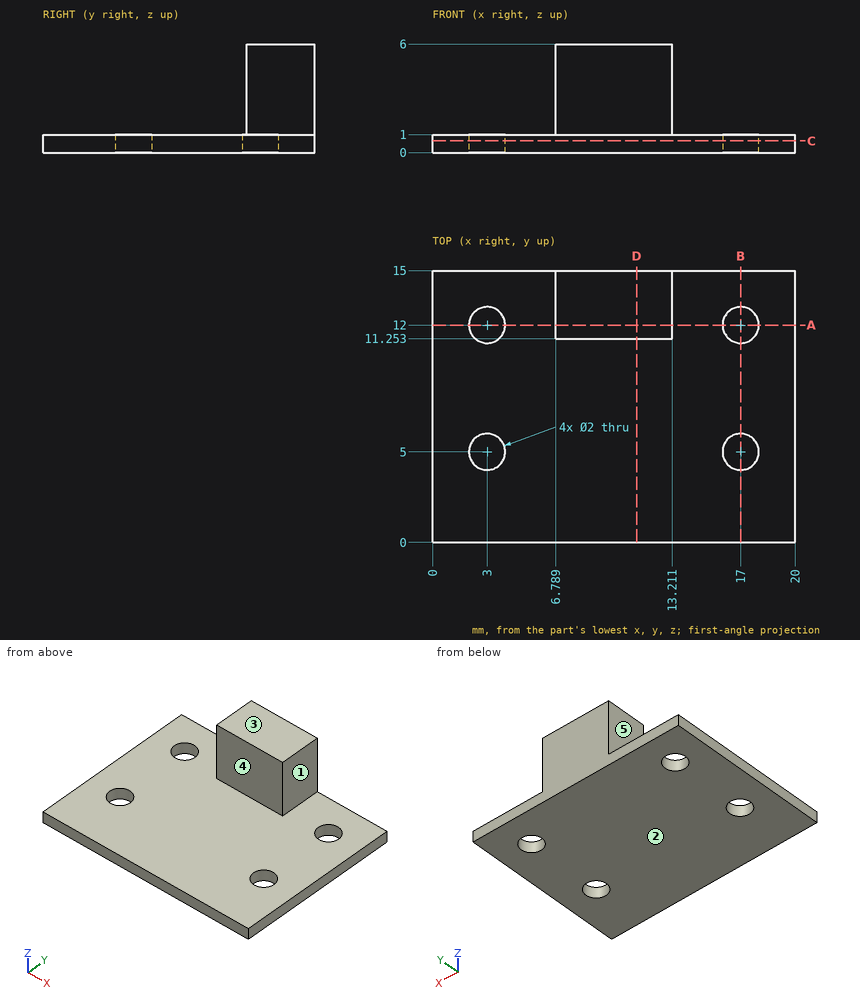
Input: dimensioned drawing with shaded views. Units: mm. Origin: part minimum x, y, z. A direction names the side the tool comes from. Round coordinates to 2 decimals unless told otherwise and drop trailing zeros. Order: outer loops, then holes, each group sorted by start corner. A loop starts at its lowest first (then second) coordinate and runs counter-clockwise, first axis right, second up. Notation, with made-up numbers: (48.5, -35.5) -> (53.5, -35.5) arc R8 cw to (53.5, -31.5) -> close; hole circle Ø7 at (55.5, 41). An arc over 180 degrees is marked (long way). Put each result on its own line as item: value. Start each with the question number.
Q1. First-contact query: pin 1 (1.5 mm diameter, centred on x = 11, z = 3, fed in from -Y); pin 2 (7.5 mm diameter, centred on x = 13, y = 5, fed in from +Z); pin 3 (1.1 mm diameter, centred on y = 13, z = 4, fed in from -X); pin 4 (1.2 mm diameter, centred on x = 17, y = 12, fed in from -Z) (3 decimals). Flat tips, straight axial feed; report the tip coordinate or a pass-through.
Q2. Section D-D on x = 11.25. Return the cut outline in (y, z).
Q3. Line query: probe 1 along Y at (x, z) = (17, 0.65); probe 2 along Z at (x, y) = (11.5, 5.25); probe 3 along Y at (x, z) = (11, 1.15). Output: solid intervals per line, ascending.
Q4. Reachability of the marked faces 1, 2, 3, 4 and 5 from +Z, -Z, +X, -X, +Y, -Y: full face, straight path, thin tool, end or side. Return the list, or none.
Q5. Section A-A on y = 12. Return the cut outline in (x, z).
Q6. Section B-B on x = 17. Return the cut outline in (y, z), and give its area (3 significant figures).
Q7. Section C-C on z = 0.65. Return the cut outline in (x, y).
Ans:
1. pin 1: stops at y = 11.25
1. pin 2: stops at z = 1
1. pin 3: stops at x = 6.79
1. pin 4: passes through
2. outline: (0, 0) -> (15, 0) -> (15, 6) -> (11.25, 6) -> (11.25, 1) -> (0, 1) -> close
3. probe 1: y = 0 to 4, 6 to 11, 13 to 15
3. probe 2: z = 0 to 1
3. probe 3: y = 11.25 to 15
4. face 1: +Z, +X, +Y, -Y
4. face 2: -Z, +X, -X, +Y, -Y
4. face 3: +Z, +X, -X, +Y, -Y
4. face 4: +Z, +X, -X, -Y
4. face 5: +Z, -X, +Y, -Y
5. outline: (0, 0) -> (2, 0) -> (2, 1) -> (0, 1) -> close; (4, 0) -> (16, 0) -> (16, 1) -> (13.21, 1) -> (13.21, 6) -> (6.79, 6) -> (6.79, 1) -> (4, 1) -> close; (18, 0) -> (20, 0) -> (20, 1) -> (18, 1) -> close
6. outline: (0, 0) -> (4, 0) -> (4, 1) -> (0, 1) -> close; (6, 0) -> (11, 0) -> (11, 1) -> (6, 1) -> close; (13, 0) -> (15, 0) -> (15, 1) -> (13, 1) -> close
6. area: 11.0 mm2
7. outline: (0, 0) -> (20, 0) -> (20, 15) -> (0, 15) -> close; hole circle Ø2 at (3, 5); hole circle Ø2 at (3, 12); hole circle Ø2 at (17, 5); hole circle Ø2 at (17, 12)
